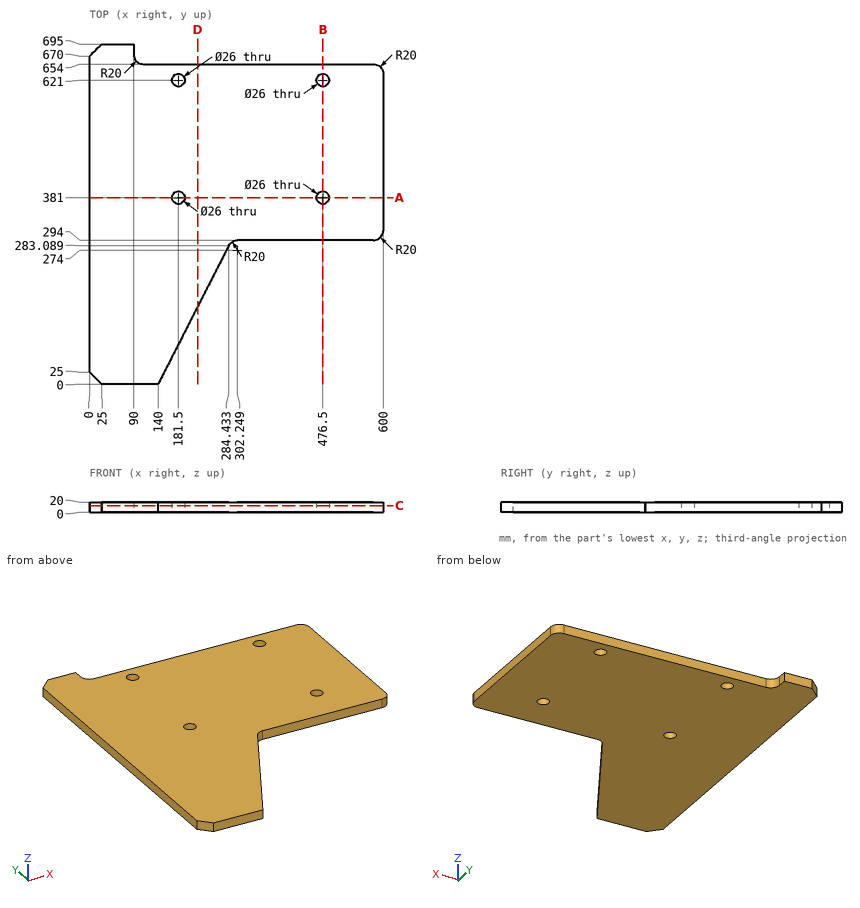
Here's the drawing with two shaded views (mm, measured from the low corner). I have some questions. Round coordinates to 2 decimals unless told otherwise and drop trailing zeros. Write each loop counter-clockwise with the first axis right and the second up, starting at its lowest first coordinate (ties: lowest second). Pieces come first, ordered by that corner, then holes. Notation, with made-up numbers: M -14.75,53.25 L 33.25,53.25 A21 cw 33.25,85.25 Z; hole C 22.25,-0.5 d9. An arc over 180 degrees is marked long. Answer in a Markdown table with one row per item. Add a question column.
Q1. Imagine slicing it at B-B (x = 476.5). Please give me the cut outline in (y, z).
Q2. Imagine slicing it at A-A (y = 381). Please give me the cut outline in (x, z), then the cut area to 3 significant figures.
Q3. Will these pins go through, and if not, where does the flat tip stop? pin 1 Ø10 at (x, z) = (309.5, 11.5) entering from +Y; pin 2 Ø2 at (x, z) = (494, 4) entering from -Y; pin 3 Ø15.5 at (x, y) = (181.5, 381) entering from +Z.
Q4. Imagine slicing it at C-C (z = 13). Please give me the cut outline in (x, y).
Q5. Imagine slicing it at D-D (x = 221). Please give me the cut outline in (y, z).
Q6. If I drill on line 1 (Y direction, x = 476.5, z = 13.75); line 2 (X direction, y = 621, z = 8.25); line 3 (Y direction, x = 181.5, z = 14.5), over which ranges is the centre line in solid material (lowest first)? Write a range as from..to.
Values:
| question | item | result |
|---|---|---|
| 1 | outline | M 294,0 L 368,0 L 368,20 L 294,20 Z; M 394,0 L 608,0 L 608,20 L 394,20 Z; M 634,0 L 654,0 L 654,20 L 634,20 Z |
| 2 | outline | M 0,0 L 168.5,0 L 168.5,20 L 0,20 Z; M 194.5,0 L 463.5,0 L 463.5,20 L 194.5,20 Z; M 489.5,0 L 600,0 L 600,20 L 489.5,20 Z |
| 2 | area | 11,000 mm^2 |
| 3 | pin 1 | y = 654 |
| 3 | pin 2 | y = 294 |
| 3 | pin 3 | through |
| 4 | outline | M 0,25 L 25,0 L 140,0 L 284.43,283.09 A20 cw 302.25,294 L 580,294 A20 ccw 600,314 L 600,634 A20 ccw 580,654 L 110,654 A20 cw 90,674 L 90,695 L 25,695 L 0,670 Z; hole C 181.5,381 d26; hole C 181.5,621 d26; hole C 476.5,381 d26; hole C 476.5,621 d26 |
| 5 | outline | M 158.76,0 L 654,0 L 654,20 L 158.76,20 Z |
| 6 | line 1 | 294..368, 394..608, 634..654 |
| 6 | line 2 | 0..168.5, 194.5..463.5, 489.5..600 |
| 6 | line 3 | 81.34..368, 394..608, 634..654 |
